from build123d import *

# Parameters (mm, degrees)
SKETCH_1_W          = 60
SKETCH_1_H          = 60
EXTRUDE_1_DEPTH     = 60
SKETCH_2_R          = 4
EXTRUDE_2_DEPTH     = 12
SKETCH_3_W          = 60
SKETCH_3_H          = 60
SKETCH_3_W_2        = 58
SKETCH_3_H_2        = 58
CUT_EXTRUDE_1_DEPTH = 7
FILLET_1_R          = 5
CHAMFER_1_SIZE      = 1
FILLET_2_R          = 5
SKETCH_5_W          = 28
SKETCH_5_H          = 38
EXTRUDE_3_DEPTH     = 24
SKETCH_6_W          = 44.228024493
SKETCH_6_H          = 29.890039758
SKETCH_6_R          = 7.083561646
CUT_EXTRUDE_2_DEPTH = 4
CUT_EXTRUDE_2_DRAFT = -30
CUT_EXTRUDE_3_DEPTH = 79.847954951


with BuildPart() as part:
    # 草图1 → 凸台-拉伸1 (new body)
    with BuildSketch(Plane.XY):
        Rectangle(SKETCH_1_W, SKETCH_1_H)
    extrude(amount=EXTRUDE_1_DEPTH)

    # 草图2 → 凸台-拉伸2 (add)
    with BuildSketch(Plane.XY.offset(60)):
        with Locations(Location((0, 0, 0), (0, 0, 180))):
            Circle(SKETCH_2_R)
    extrude(amount=EXTRUDE_2_DEPTH)

    # 草图3 → 切除-拉伸1 (cut)
    with BuildSketch(Plane(origin=(0, 0, 0), x_dir=(-1, 0, 0), z_dir=(0, 0, -1))):
        Rectangle(SKETCH_3_W, SKETCH_3_H)
        Rectangle(SKETCH_3_W_2, SKETCH_3_H_2, mode=Mode.SUBTRACT)
    extrude(amount=-CUT_EXTRUDE_1_DEPTH, mode=Mode.SUBTRACT)

    # 圆角1
    fillet_1_edges = [part.edges().sort_by_distance(p)[0] for p in [
        (-29, -29, 3.5),
        (29, -29, 3.5),
        (29, 29, 3.5),
        (-29, 29, 3.5),
    ]]
    fillet(fillet_1_edges, radius=FILLET_1_R)

    # 倒角1
    chamfer_1_edges = [part.edges().sort_by_distance(p)[0] for p in [
        (-29, 0, 0),
        (0, -29, 0),
        (0, 29, 0),
        (29, 0, 0),
        (27.535533906, 27.535533906, 0),
        (27.535533906, -27.535533906, 0),
        (-27.535533906, -27.535533906, 0),
        (-27.535533906, 27.535533906, 0),
    ]]
    chamfer(chamfer_1_edges, length=CHAMFER_1_SIZE)

    # 圆角2
    fillet_2_edges = [part.edges().sort_by_distance(p)[0] for p in [
        (30, -30, 33.5),
        (-30, -30, 33.5),
        (-30, 30, 33.5),
        (30, 30, 33.5),
    ]]
    fillet(fillet_2_edges, radius=FILLET_2_R)

    # 草图5 → 凸台-拉伸3 (add)
    with BuildSketch(Plane(origin=(0, 30, 0), x_dir=(1, 0, 0), z_dir=(0, 1, 0))):
        with Locations((0, -38)):
            Rectangle(SKETCH_5_W, SKETCH_5_H)
    extrude(amount=EXTRUDE_3_DEPTH)


with BuildPart() as cut_extrude_2_tool:
    # 草图6 → 切除-拉伸2 (with draft: the straight prism first)
    with BuildSketch(Plane(origin=(0, 0, 19), x_dir=(-1, 0, 0), z_dir=(0, 0, -1))):
        with Locations((-0.478057726, 44.945019879)):
            Rectangle(SKETCH_6_W, SKETCH_6_H)
        with Locations((0, 42)):
            Circle(SKETCH_6_R, mode=Mode.SUBTRACT)
    extrude(amount=-CUT_EXTRUDE_2_DEPTH)
    # 切除-拉伸2: the draft: its side faces are tilted about the plane it starts from
    cut_extrude_2_sides = [cut_extrude_2_tool.faces().sort_by_distance(p)[0] for p in [
        (22.592069973, 44.945019879, 21),
        (0.478057727, 30, 21),
        (-21.63595452, 44.945019879, 21),
        (0.478057727, 59.890039758, 21),
        (7.083561646, 42, 21),
    ]]
    draft(cut_extrude_2_sides, Plane(origin=(0, 0, 19), x_dir=(-1, 0, 0), z_dir=(0, 0, -1)), CUT_EXTRUDE_2_DRAFT)


with BuildPart() as part_1:
    add(part.part)

    # 切除-拉伸2: cut by cut_extrude_2_tool
    add(cut_extrude_2_tool.part, mode=Mode.SUBTRACT)

    # 草图7 → 切除-拉伸3 (cut, through all)
    with BuildSketch(Plane(origin=(0, 0, 23), x_dir=(-1, 0, 0), z_dir=(0, 0, -1))):
        Polygon((-14, 51.383198576), (-9.015728145, 54), (9.073415265, 54), (14, 51.383198576), (16.492135927, 52.691599288), (15.246067964, 56.551525264), (-18.004122386, 56.551525264), align=None)
    extrude(amount=-CUT_EXTRUDE_3_DEPTH, mode=Mode.SUBTRACT)


solid = part_1.part
Can you work these out from the model? Positions are in its coordinate system, mm. A direction names the side the tool comes from. Round coordinates to 2 decimals unless told otherwise and drop trailing zeros. Loops run counter-clockwise (first coordinate to the right, second up) from the corner with the lowest first, then second, coordinate; pieces in that order, holes last. Notation, with made-up numbers: (-28.75, -18.5) - (-19.75, -18.5) arc R28 ccw to (-19.75, 13.5) - close; hole circle Ø3 at (-1.75, 77). An arc over 180 degrees is marked (long way). Write item = value, one per line. Start each with the question number.
(1) If we section it at D-D (x = -18): Please give me the cut outline in (y, z).
(2) If I drill on probe 1 along Z at (x, y) = (-14, 0); probe 2 along X at (y, z) = (48, 48); probe 3 along Y at (x, z) = (-6, 17.5), over which ranges is the centre line in solid material (lowest first)? Write a range as [from, to].
(3) If we section it at B-B (z = 25.5): Please give me the cut outline in (x, y), and give its area (3 significant figures).
(4) For faces 5 (the face through (0, 42, 57)), 6 (the face through (0, 29, 4)), 7 (the face through (0, -29, 4)), which set-ups out of +Z, -Z, +X, -X, +Y, -Y let a thin tool reach every point of the face, with its end or its side?
(5) For P1, Ø3, axis at x = 12, y = 33, coming from the +Z side; P2, Ø5, axis at y = 7, z = 4, coming from the +X side; P3, Ø3, axis at x = -9, z = 4.5, coming from the +Y side, each with a flat end and sliding along its axis, tell me the tip position at first contact or that it passes through.
(6) If we section it at C-C (y = 42): Please give me the cut outline in (x, z), and give its area (3 significant figures).
(7) If we section it at A-A (x = 0): Please give me the cut outline in (y, z).
(8) If we mould it in two halves opening along Y, with no side actions, what happens to faces 1 (the face through (0, 0, 72)), 2 (the face through (0.196, 31.139, 20.972)), 3 (the face through (6, 51, 23)), 4 (the face through (-28, -29, 34))? For each: released by +Y, released by -Y, zero draft, split by the parting line, or undercut.
Ans:
q1.outline = (-30, 7) - (-29, 7) - (-29, 1) - (-28, 0) - (28, 0) - (29, 1) - (29, 7) - (30, 7) - (30, 60) - (-30, 60) - close
q2.probe_1 = [0, 60]
q2.probe_2 = [-14, 14]
q2.probe_3 = [-30, 30]
q3.outline = (-30, -25) arc R5 ccw to (-25, -30) - (25, -30) arc R5 ccw to (30, -25) - (30, 25) arc R5 ccw to (25, 30) - (14, 30) - (14, 51.38) - (9.02, 54) - (-9.07, 54) - (-14, 51.38) - (-14, 30) - (-25, 30) arc R5 ccw to (-30, 25) - close
q3.area = 4,240 mm²
q4.face_5 = +Z, +X, -X, +Y
q4.face_6 = -Z, +X, -X, +Y
q4.face_7 = -Z, +X, -X, -Y
q5.P1 = 57
q5.P2 = 29
q5.P3 = 29
q6.outline = (-14, 23) - (-9.39, 23) - (-7.08, 19) - (7.08, 19) - (9.39, 23) - (14, 23) - (14, 57) - (-14, 57) - close
q6.area = 1,020 mm²
q7.outline = (-30, 7) - (-29, 7) - (-29, 1) - (-28, 0) - (28, 0) - (29, 1) - (29, 7) - (30, 7) - (30, 19) - (32.31, 23) - (32.61, 23) - (34.92, 19) - (49.08, 19) - (51.39, 23) - (54, 23) - (54, 57) - (30, 57) - (30, 60) - (4, 60) - (4, 72) - (-4, 72) - (-4, 60) - (-30, 60) - close
q8.face_1 = zero draft
q8.face_2 = undercut
q8.face_3 = undercut
q8.face_4 = released by -Y
